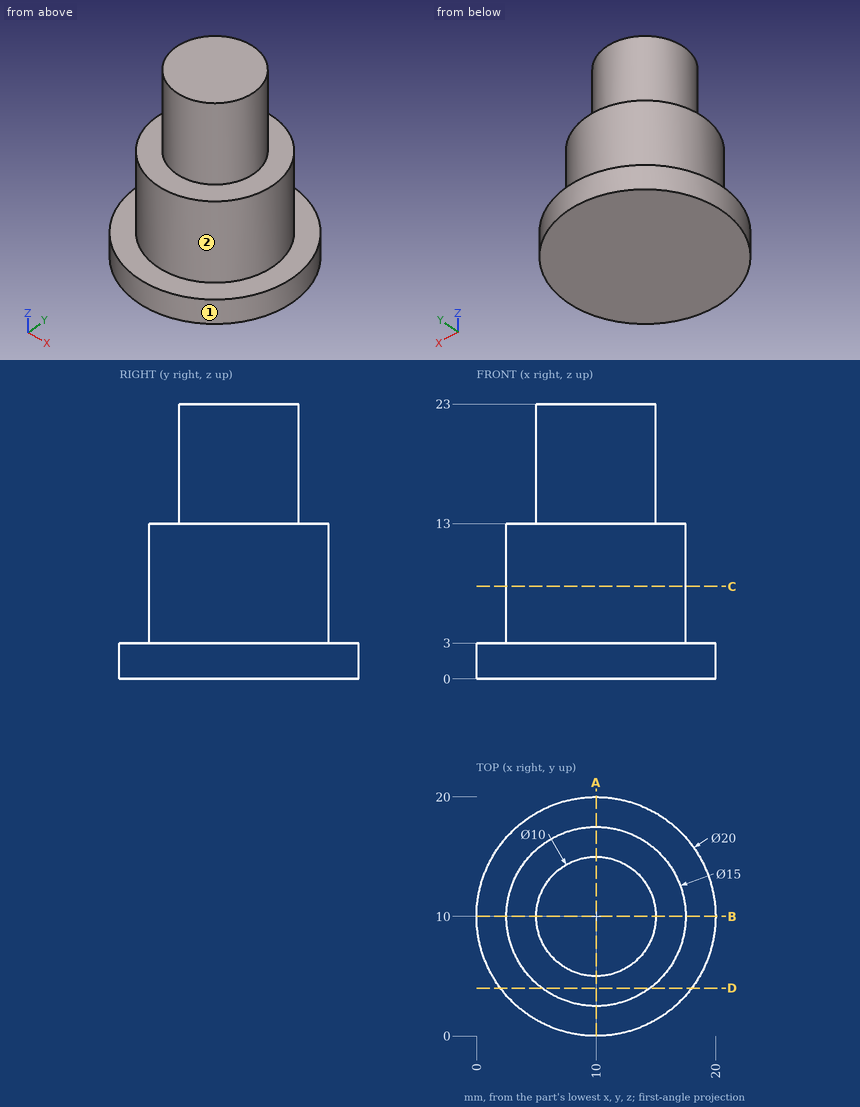
Job drawing, mm, ordinate dimensions from the low corner. One solid piece. A direction names the side the tool comes from. Coordinates: 2 decimals unless noted, no trailing zeros. Order: outer loops, then holes, each group sorted by start corner. A loop starts at its lowest first (then second) coordinate and runs counter-clockwise, first axis right, second up. Notation, with made-up numbers: M 36,50 L 94,50 A34 ccw 94,87 Z; hole C 87.25,3 d7. An arc over 180 degrees is marked long. One line per question, with ' | ' between items.
Q1. Pin check, flat tips, straight feed: P1, Ø12, axis at x = 13.5, z = 3.5, coming from the +Y side; P2, Ø1, axis at y = 7.5, z = 19.5, coming from the -X side; P3, Ø6, axis at x = 9, z = 13, coming from the -Y side; P4, Ø1, axis at x = 6.5, z = 5.5, coming from the +Y side. Stop position of each tip, or through.
A:
P1: stops at y = 20 | P2: stops at x = 5.42 | P3: stops at y = 2.5 | P4: stops at y = 16.87
Q2. Slice it at D-D (y = 4). Give the cut face in (x, z).
A:
outline: M 2,0 L 18,0 L 18,3 L 14.5,3 L 14.5,13 L 5.5,13 L 5.5,3 L 2,3 Z
Q3. Slice it at A-A (x = 10). Give the cut face in (y, z).
A:
outline: M 0,0 L 20,0 L 20,3 L 17.5,3 L 17.5,13 L 15,13 L 15,23 L 5,23 L 5,13 L 2.5,13 L 2.5,3 L 0,3 Z
Q4. 3-axis set-ups, long thin cutter, end or side, ignore diameter. For the marked faces 1 and 2: which of +Z, -Z, +X, -X, +Y, -Y reach the whole face in a straight line?
A:
face 1: +Z, -Z | face 2: +Z
Q5. Drill centre lines: line 1 (Z direction, x = 9.25, y = 1.75); line 2 (X direction, y = 9.75, z = 12); line 3 (Z direction, x = 11, y = 4.75). Where is each one in solid material? Low to high.
A:
line 1: z = 0 to 3 | line 2: x = 2.5 to 17.5 | line 3: z = 0 to 13
Q6. Slice it at C-C (z = 7.75). Give the cut face in (x, y), and give its area (3 significant figures).
A:
outline: C 10,10 d15 | area: 177 mm^2
